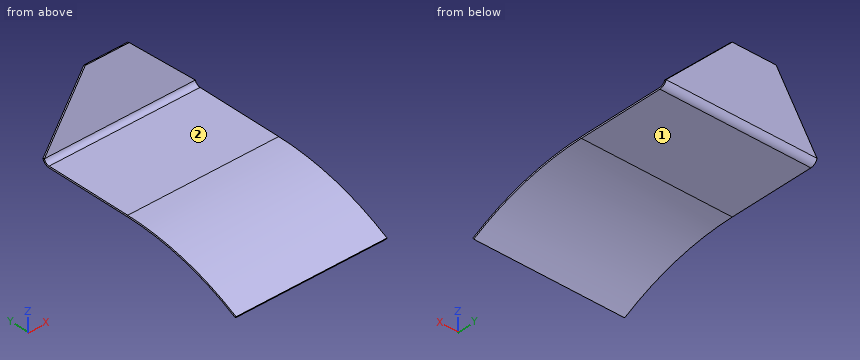
from build123d import *

# Parameters (mm, degrees)
BOSS_EXTRUDE1_DEPTH = 70.5
CHAMFER1_SIZE       = 50


with BuildPart() as part:
    # Sketch1 → Boss-Extrude1 (new, symmetric)
    with BuildSketch(Plane(origin=(0, 0, 0), x_dir=(0, 0, -1), z_dir=(1, 0, 0))):
        with BuildLine():
            ThreePointArc((-230.8, 80.4), (-231.833233299, 83.443807145), (-234.505904774, 85.229629131))
            Line((-234.505904774, 85.229629131), (-282.802196089, 98.170581387))
            Line((-282.802196089, 98.170581387), (-282.413967521, 99.619470126))
            Line((-282.413967521, 99.619470126), (-234.117676207, 86.678517871))
            ThreePointArc((-234.117676207, 86.678517871), (-230.643203288, 84.356949289), (-229.3, 80.4))
            Line((-229.3, 80.4), (-229.3, 0))
            ThreePointArc((-229.3, 0), (-222.145797616, -56.830754012), (-201.129615338, -110.115247964))
            Line((-201.129615338, -110.115247964), (-202.445334583, -110.83558321))
            ThreePointArc((-202.445334583, -110.83558321), (-223.598997339, -57.202520828), (-230.8, 0))
            Line((-230.8, 0), (-230.8, 80.4))
        make_face()
    extrude(amount=BOSS_EXTRUDE1_DEPTH, both=True)

    # Chamfer1
    chamfer1_edges = [part.edges().sort_by_distance(p)[0] for p in [
        (-70.5, 98.895025756, 282.608081805),
        (70.5, 98.895025756, 282.608081805),
    ]]
    chamfer(chamfer1_edges, length=CHAMFER1_SIZE)


solid = part.part
Here's how the part is built. I have some questions about the finished solid (model axes, mm). Face numbers are marked on the shaded views. A direction names the side the tool comes from. Round coordinates to 2 decimals unless told otherwise and drop trailing zeros. Order: outer loops, then holes, each group sorted by start corner. A loop starts at its lowest first (then second) coordinate and runs counter-clockwise, first axis right, second up. Notation, with made-up numbers: M -7,8.25 L 6,8.25 A23 cw 6,26.25 Z; hole C 30,84 d7. An arc over 180 degrees is marked long. Return JSON: item names as keys, results as strings. Group by question number.
1. On a 3-axis mill with a long thin cutter (end or side, diameter ignored), from which of +Z, -Z, +X, -X, +Y, -Y can I reach the whole of each face in a straight line? I mean the marked faces 1 and 2. Say none if no direction works.
2. If we section it at B-B on z = 221: List the corners of the cut face in (x, y) for me, then the cut area to 3 significant figures.
3. Please list where these lines run through material, in increasing order: probe 1 along Z at (x, y) = (-9.5, 46.5); probe 2 along Z at (x, y) = (8, -4); probe 3 along Y at (x, z) = (24.5, 270.5).
4. If we section it at A-A on y = 48.5: List the corners of the cut face in (x, z) for me.
5. I'm going to push flat-ended pins straight in: pin 1 Ø4 at (x, y) = (-21, -52.5) entering from +Z; pin 2 Ø4 at (x, z) = (1, 236) entering from -Y; pin 3 Ø10 at (x, z) = (15.5, 267.5) entering from -Y. Where does each tip first touch, or does it pass through?
Reply:
{
 "1": {"face 1": "-Z, +X, -X, +Y", "face 2": "+Z, +X, -X, -Y"},
 "2": {"outline": "M -70.5,-66.54 L 70.5,-66.54 L 70.5,-61.14 L -70.5,-61.14 Z", "area": "762 mm^2"},
 "3": {"probe 1": "229.3 to 230.8", "probe 2": "229.27 to 230.77", "probe 3": "94.87 to 96.43"},
 "4": {"outline": "M -70.5,229.3 L 70.5,229.3 L 70.5,230.8 L -70.5,230.8 Z"},
 "5": {"pin 1": "z = 225.21", "pin 2": "y = 85.06", "pin 3": "y = 92.73"}
}
